```python
from build123d import *

# Parameters (mm, degrees)
SKETCH1_R           = 4
BOSS_EXTRUDE1_DEPTH = 6
SKETCH3_R           = 6.5
CUT_EXTRUDE2_DEPTH  = 3
CUT_EXTRUDE3_START  = -1
SKETCH4_R           = 6.5
SKETCH4_R_2         = 5
CUT_EXTRUDE3_DEPTH  = 1
SKETCH5_W           = 15
SKETCH5_H           = 3
BOSS_EXTRUDE2_DEPTH = 6
SKETCH6_R           = 1.2
CUT_EXTRUDE7_DEPTH  = 17
FILLET3_R           = 2.5
SKETCH7_R           = 2.2
CUT_EXTRUDE8_DEPTH  = 4


with BuildPart() as part:
    # Sketch1 → Boss-Extrude1 (new body)
    with BuildSketch(Plane.XY):
        Polygon((7.5, 0), (7.5, 7.5), (-7.5, 7.5), (-7.5, -7.5), (7.5, -7.5), align=None)
        Circle(SKETCH1_R, mode=Mode.SUBTRACT)
    extrude(amount=BOSS_EXTRUDE1_DEPTH)

    # Sketch3 → Cut-Extrude2 (cut)
    with BuildSketch(Plane(origin=(0, 0, 0), x_dir=(-1, 0, 0), z_dir=(0, 0, -1))):
        Circle(SKETCH3_R)
    extrude(amount=-CUT_EXTRUDE2_DEPTH, mode=Mode.SUBTRACT)

    # Sketch4 → Cut-Extrude3 (cut)
    with BuildSketch(Plane.XY.offset(6).offset(CUT_EXTRUDE3_START)):
        with Locations(Location((0, 0, 0), (0, 0, 180))):
            Circle(SKETCH4_R)
        Circle(SKETCH4_R_2, mode=Mode.SUBTRACT)
    extrude(amount=CUT_EXTRUDE3_DEPTH, mode=Mode.SUBTRACT)

    # Sketch5 → Boss-Extrude2 (add)
    with BuildSketch(Plane(origin=(0, 0, 0), x_dir=(-1, 0, 0), z_dir=(0, 0, -1))):
        with Locations((0, -9)):
            Rectangle(SKETCH5_W, SKETCH5_H)
        with Locations((0, 9)):
            Rectangle(SKETCH5_W, SKETCH5_H)
    extrude(amount=-BOSS_EXTRUDE2_DEPTH)

    # Sketch6 → Cut-Extrude7 (cut)
    with BuildSketch(Plane(origin=(0, 0, 0), x_dir=(-1, 0, 0), z_dir=(0, 0, -1))):
        with Locations((5, 8)):
            Circle(SKETCH6_R)
        with Locations((-5, 8)):
            Circle(SKETCH6_R)
        with Locations((-5, -8)):
            Circle(SKETCH6_R)
        with Locations((5, -8)):
            Circle(SKETCH6_R)
    extrude(amount=-CUT_EXTRUDE7_DEPTH, mode=Mode.SUBTRACT)

    # Fillet3
    fillet3_edges = [part.edges().sort_by_distance(p)[0] for p in [
        (-7.5, -10.5, 3),
        (7.5, -10.5, 3),
        (7.5, 10.5, 3),
        (-7.5, 10.5, 3),
    ]]
    fillet(fillet3_edges, radius=FILLET3_R)

    # Sketch7 → Cut-Extrude8 (cut)
    with BuildSketch(Plane(origin=(0, 0, 0), x_dir=(-1, 0, 0), z_dir=(0, 0, -1))):
        with Locations((-5, -8)):
            Circle(SKETCH7_R)
        with Locations((-5, 8)):
            Circle(SKETCH7_R)
        with Locations((5, 8)):
            Circle(SKETCH7_R)
        with Locations((5, -8)):
            Circle(SKETCH7_R)
    extrude(amount=-CUT_EXTRUDE8_DEPTH, mode=Mode.SUBTRACT)


solid = part.part
```
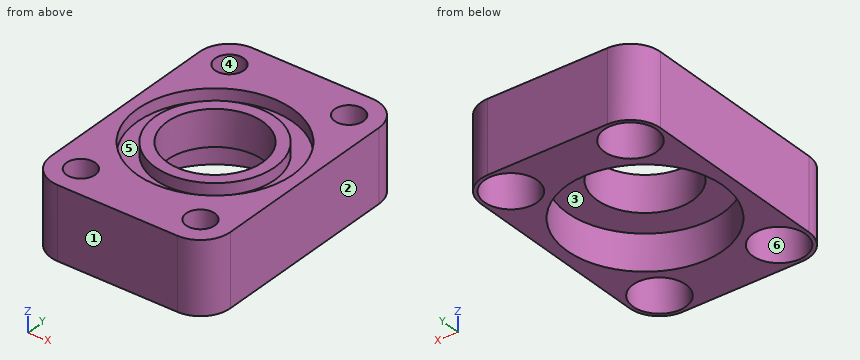
Build history of the part. All positions in model axes, mm. Face numbers are marked on the shaded views. A direction names the side the tool comes from. Coordinates: 2 decimals unless noted, no trailing zeros. Order: outer loops, then holes, each group sorted by start corner. A loop starts at its lowest first (then second) coordinate and runs counter-clockwise, first axis right, second up.
Item 1: Tool access for the marked faces 4, 5 and 6: list every direction of +Z, -Z, +X, -X, +Y, -Y with a clear straight run to the whole face (end or side of a thin tool).
Filled in:
face 4: +Z, -Z
face 5: +Z
face 6: -Z
Item 2: Saw through at C-C on z = 2.15. List the corners of the cut face in (x, y), then the cut area to 3 significant figures.
Filled in:
outline: (-7.5, -8) arc R2.5 ccw to (-5, -10.5) - (5, -10.5) arc R2.5 ccw to (7.5, -8) - (7.5, 8) arc R2.5 ccw to (5, 10.5) - (-5, 10.5) arc R2.5 ccw to (-7.5, 8) - close; hole circle Ø4.4 at (-5, -8); hole circle Ø4.4 at (-5, 8); hole circle Ø13 at (0, 0); hole circle Ø4.4 at (5, -8); hole circle Ø4.4 at (5, 8)
area: 116 mm2
Item 3: Drop flat-ended pins along their axis: pin 1 Ø2.5 at (x, y) = (5, 8) entering from -Z; pin 2 Ø6.5 at (x, y) = (0, -3) entering from -Z; pin 3 Ø2 at (x, y) = (5, -8) entering from +Z. Give the stop position or say it passes through.
Filled in:
pin 1: stops at z = 4
pin 2: stops at z = 3
pin 3: passes through
Item 4: Mould opens along Y. For the marked faces 1, 2 and 3 say: released by +Y, released by -Y, zero draft, split by the parting line, or undercut.
Filled in:
face 1: released by -Y
face 2: zero draft
face 3: undercut
Item 5: Drill centre lines: L1, parallel to Y at x = 0, z = 2.05; L2, parallel to X at y = -8.5, z = 2.6; L3, parallel to Y at x = 4.5, z = 1.7. Where is each one in solid material? Low to high.
Filled in:
L1: y = -10.5 to -6.5, 6.5 to 10.5
L2: x = -7.45 to -7.14, -2.86 to 2.86, 7.14 to 7.45
L3: y = -10.5 to -10.14, -5.86 to -4.69, 4.69 to 5.86, 10.14 to 10.5
Item 6: Saw through at D-D on x = -5.75. List the corners of the cut face in (y, z).
Filled in:
outline: (-10.38, 0) - (-10.07, 0) - (-10.07, 4) - (-8.94, 4) - (-8.94, 6) - (-10.38, 6) - close; (-7.06, 4) - (-5.93, 4) - (-5.93, 0) - (-3.03, 0) - (-3.03, 3) - (3.03, 3) - (3.03, 0) - (5.93, 0) - (5.93, 4) - (7.06, 4) - (7.06, 6) - (3.03, 6) - (3.03, 5) - (-3.03, 5) - (-3.03, 6) - (-7.06, 6) - close; (8.94, 4) - (10.07, 4) - (10.07, 0) - (10.38, 0) - (10.38, 6) - (8.94, 6) - close
Item 7: Saw through at B-B on x = 0. List the corners of the cut face in (y, z).
Filled in:
outline: (-10.5, 0) - (-6.5, 0) - (-6.5, 3) - (-4, 3) - (-4, 6) - (-5, 6) - (-5, 5) - (-6.5, 5) - (-6.5, 6) - (-10.5, 6) - close; (4, 3) - (6.5, 3) - (6.5, 0) - (10.5, 0) - (10.5, 6) - (6.5, 6) - (6.5, 5) - (5, 5) - (5, 6) - (4, 6) - close
Item 8: Saw through at A-A on y = 0. List the corners of the cut face in (x, z).
Filled in:
outline: (-7.5, 0) - (-6.5, 0) - (-6.5, 3) - (-4, 3) - (-4, 6) - (-5, 6) - (-5, 5) - (-6.5, 5) - (-6.5, 6) - (-7.5, 6) - close; (4, 3) - (6.5, 3) - (6.5, 0) - (7.5, 0) - (7.5, 6) - (6.5, 6) - (6.5, 5) - (5, 5) - (5, 6) - (4, 6) - close
